```python
from build123d import *

# Parameters (mm, degrees)
SKETCH1_R           = 15
BOSS_EXTRUDE1_DEPTH = 65
SKETCH2_R           = 14
BOSS_EXTRUDE2_DEPTH = 260
SKETCH3_W           = 22.007775422
SKETCH3_H           = 2
CUT_EXTRUDE1_DEPTH  = 22
CIRPATTERN1_COUNT   = 4
SKETCH4_R           = 10.5
BOSS_EXTRUDE3_DEPTH = 30
SKETCH5_R           = 10.3
BOSS_EXTRUDE4_DEPTH = 10
SKETCH6_R           = 10.5
BOSS_EXTRUDE5_DEPTH = 16
CHAMFER1_SIZE       = 8
CHAMFER1_SIZE2      = 1
SKETCH8_R           = 7.5
BOSS_EXTRUDE6_DEPTH = 30
BOSS_EXTRUDE7_START = -8
SKETCH11_R          = 21
SKETCH11_R_2        = 15
BOSS_EXTRUDE7_DEPTH = 8
SKETCH13_R          = 19
CUT_EXTRUDE4_DEPTH  = 373
SKETCH14_R          = 8.4
BOSS_EXTRUDE8_DEPTH = 10
CHAMFER3_SIZE       = 1
SKETCH16_R          = 1.75
CUT_EXTRUDE5_DEPTH  = 43.213741838
CIRPATTERN3_COUNT   = 4


with BuildPart() as part:
    # Sketch1 → Boss-Extrude1 (new body)
    with BuildSketch(Plane(origin=(0, 0, 0), x_dir=(1, 0, 0), z_dir=(0, 1, 0))):
        with Locations(Location((0, 0, 0), (0, 0, 270))):
            Circle(SKETCH1_R)
    extrude(amount=BOSS_EXTRUDE1_DEPTH)

    # Sketch2 → Boss-Extrude2 (add)
    with BuildSketch(Plane.XZ):
        with Locations(Location((0, 0, 0), (0, 0, 90))):
            Circle(SKETCH2_R)
    extrude(amount=BOSS_EXTRUDE2_DEPTH)

    # Sketch3 → Cut-Extrude1 (cut)
    with BuildSketch(Plane.XZ.offset(260)):
        with Locations((0, -14)):
            Rectangle(SKETCH3_W, SKETCH3_H)
        with Locations((0, 14)):
            Rectangle(SKETCH3_W, SKETCH3_H)
    cut_extrude1 = extrude(amount=-CUT_EXTRUDE1_DEPTH, mode=Mode.SUBTRACT)

    # CirPattern1: Cut-Extrude1 ×4 about axis
    cirpattern1_axis = Axis((0, -260, 0), (0, 1, 0))
    for i in range(1, CIRPATTERN1_COUNT):
        add(cut_extrude1.rotate(cirpattern1_axis, i * 360 / CIRPATTERN1_COUNT), mode=Mode.SUBTRACT)

    # Sketch4 → Boss-Extrude3 (add)
    with BuildSketch(Plane.XZ.offset(260)):
        with Locations(Location((0, 0, 0), (0, 0, 270))):
            Circle(SKETCH4_R)
    extrude(amount=BOSS_EXTRUDE3_DEPTH)

    # Sketch5 → Boss-Extrude4 (add)
    with BuildSketch(Plane.XZ.offset(290)):
        with Locations(Location((0, 0, 0), (0, 0, 270))):
            Circle(SKETCH5_R)
    extrude(amount=BOSS_EXTRUDE4_DEPTH)

    # Sketch6 → Boss-Extrude5 (add)
    with BuildSketch(Plane.XZ.offset(300)):
        with Locations(Location((0, 0, 0), (0, 0, 270))):
            Circle(SKETCH6_R)
    extrude(amount=BOSS_EXTRUDE5_DEPTH)

    # Chamfer1
    chamfer1_edges = [part.edges().sort_by_distance(p)[0] for p in [
        (0, -316, 10.5),
    ]]
    chamfer1_side = [part.faces().sort_by_distance(p)[0] for p in [
        (0, -308, 10.5),
    ]]
    chamfer(chamfer1_edges, length=CHAMFER1_SIZE, length2=CHAMFER1_SIZE2, reference=chamfer1_side[0])

    # Sketch8 → Boss-Extrude6 (add)
    with BuildSketch(Plane(origin=(0, 65, 0), x_dir=(1, 0, 0), z_dir=(0, 1, 0))):
        with Locations(Location((0, 0, 0), (0, 0, 270))):
            Circle(SKETCH8_R)
    extrude(amount=BOSS_EXTRUDE6_DEPTH)

    # Sketch11 → Boss-Extrude7 (add)
    with BuildSketch(Plane(origin=(0, 65, 0), x_dir=(1, 0, 0), z_dir=(0, 1, 0)).offset(BOSS_EXTRUDE7_START)):
        with Locations(Location((0, 0, 0), (0, 0, 270))):
            Circle(SKETCH11_R)
        with Locations(Location((0, 0, 0), (0, 0, 270))):
            Circle(SKETCH11_R_2, mode=Mode.SUBTRACT)
    extrude(amount=BOSS_EXTRUDE7_DEPTH)

    # Sketch13 → Cut-Extrude4 (cut)
    with BuildSketch(Plane.XZ.offset(316)):
        Circle(SKETCH13_R)
    extrude(amount=-CUT_EXTRUDE4_DEPTH, mode=Mode.SUBTRACT)

    # Sketch14 → Boss-Extrude8 (add)
    with BuildSketch(Plane.XZ.offset(-57)):
        with Locations(Location((0, 0, 0), (0, 0, 90))):
            Circle(SKETCH14_R)
    extrude(amount=BOSS_EXTRUDE8_DEPTH)

    # Chamfer3
    chamfer3_edges = [part.edges().sort_by_distance(p)[0] for p in [
        (0, 95, -7.5),
        (0, 47, -8.4),
    ]]
    chamfer(chamfer3_edges, length=CHAMFER3_SIZE)

    # Sketch16 → Cut-Extrude5 (cut, through all)
    with BuildSketch(Plane(origin=(0, 65, 0), x_dir=(1, 0, 0), z_dir=(0, 1, 0))):
        with Locations(Location((17.5, 0, 0), (0, 0, 270))):
            Circle(SKETCH16_R)
    cut_extrude5 = extrude(amount=-CUT_EXTRUDE5_DEPTH, mode=Mode.SUBTRACT)

    # CirPattern3: Cut-Extrude5 ×4 about axis
    cirpattern3_axis = Axis((0, 0, 0), (0, 1, 0))
    for i in range(1, CIRPATTERN3_COUNT):
        add(cut_extrude5.rotate(cirpattern3_axis, i * 360 / CIRPATTERN3_COUNT), mode=Mode.SUBTRACT)


solid = part.part
```
Verification items for the finished model (mm, model axes). A direction names the side the tool comes from. Coordinates: 2 decimals unless noted, no trailing zeros. Loops run counter-clockwise (first coordinate to the right, second up) from the corner with the lowest first, then second, coordinate; pieces in that order, holes last. Notation, with made-up numbers: (-21.75, 69) -> (8.25, 69) arc R34 cw to (8.25, 107) -> close; hole circle Ø5 at (-36.75, 48). An arc over 180 degrees is marked (long way). Answer in a Markdown table with one row per item. Add a question column.
1. Access from +Z, -Z, +X, -X, +Y, -Y to the whole of each face (thin tool, end or side, straight path). Record for faces 1 (the face through (0.33, 79.297, -7.493)), 2 (the face through (-0.228, 61.056, -19.235)), 3 (the face through (0, 57, 9)).
2. Section check D-D, the plane y = 62.5. Enter the section's corners in (x, z), then the cut area to 3 significant figures.
3. Material ranges on probe 1 along X at (y, z) = (61, 0); probe 2 along Y at (x, z) = (-10.5, 0.5); probe 3 along X at (y, z) = (61.5, -17.5), recorded low to high. Write a range as [from, to].
4. Depth check by flat-ended pin: P1, Ø3, axis at x = -7.5, z = -12, coming from the -Y side; P2, Ø10, axis at y = 85, z = -7, coming from the +X side; P3, Ø8, axis at y = 52.5, z = 10, coming from the +X side. Enter the tip coordinate at first touch or a pass-through.
5. Draft check along X on faces 4 (the face through (0, 47, 0)), 5 (the face through (19.235, 61.056, -0.228)), 6 (the face through (-2.523, 52.563, 8.012)). Enter one of: +X half, -X half, draft (parallel to the pull), parting line (faces both ways), or undercut.
6. Section check C-C, the plane z = 16.5. Enter the section's corners in (x, y), then the cut area to 3 significant figures.
7. Section check A-A, the plane z = 0. Enter the section's corners in (x, y), then the cut area to 3 significant figures.
8. Section check B-B, the plane x = 17.5. Enter the section's corners in (y, z), then the cut area to 3 significant figures.
Derived:
| question | item | result |
|---|---|---|
| 1 | face 1 | +Y |
| 1 | face 2 | +Y, -Y |
| 1 | face 3 | -Y |
| 2 | outline | circle Ø42 at (0, 0); hole circle Ø3.5 at (-17.5, 0); hole circle Ø3.5 at (0, -17.5); hole circle Ø3.5 at (0, 17.5); hole circle Ø3.5 at (17.5, 0) |
| 2 | area | 1,350 mm² |
| 3 | probe 1 | x = [-21, -19.25], [-15.75, 15.75], [19.25, 21] |
| 3 | probe 2 | y = [57, 65] |
| 3 | probe 3 | x = [-11.61, -1.75], [1.75, 11.61] |
| 4 | P1 | stops at y = 57 |
| 4 | P2 | stops at x = 7.23 |
| 4 | P3 | stops at x = 5.88 |
| 5 | face 4 | draft |
| 5 | face 5 | undercut |
| 5 | face 6 | parting line |
| 6 | outline | (-12.99, 57) -> (-1.44, 57) -> (-1.44, 65) -> (-12.99, 65) -> close; (1.44, 57) -> (12.99, 57) -> (12.99, 65) -> (1.44, 65) -> close |
| 6 | area | 185 mm² |
| 7 | outline | (-21, 57) -> (-19.25, 57) -> (-19.25, 65) -> (-21, 65) -> close; (-15.75, 57) -> (-8.4, 57) -> (-8.4, 48) -> (-7.4, 47) -> (7.4, 47) -> (8.4, 48) -> (8.4, 57) -> (15.75, 57) -> (15.75, 65) -> (7.5, 65) -> (7.5, 94) -> (6.5, 95) -> (-6.5, 95) -> (-7.5, 94) -> (-7.5, 65) -> (-15.75, 65) -> close; (19.25, 57) -> (21, 57) -> (21, 65) -> (19.25, 65) -> close |
| 7 | area | 896 mm² |
| 8 | outline | (57, -11.61) -> (65, -11.61) -> (65, -1.75) -> (57, -1.75) -> close; (57, 1.75) -> (65, 1.75) -> (65, 11.61) -> (57, 11.61) -> close |
| 8 | area | 158 mm² |
